Read the model definition and answer for the solid it produces. Units are mm, in the model's axes. A direction names the side the tool comes from. Coordinates: 2 decimals unless noted, no trailing zeros. Write each loop counter-clockwise with the first axis right and the second up, starting at its lowest first coordinate (ties: lowest second). Pieces come first, ordered by that corner, then holes. Notation, with made-up numbers: M 22.25,25.25 L 75.25,25.25 A9 ccw 75.25,34.25 Z; hole C 1.25,80 d2. An arc over 180 degrees is marked long. Write item = value, one per line.
from build123d import *

# Parameters (mm, degrees)
SKETCH_1_R                = 21
SKETCH_1_R_2              = 12.5
EXTRUDE_1_DEPTH           = 71
SKETCH_2_R                = 32.5
SKETCH_2_R_2              = 12.5
EXTRUDE_2_DEPTH           = 13
HOLE_WIZARD_1_D           = 5.5
HOLE_WIZARD_1_CBORE_D     = 10
HOLE_WIZARD_1_CBORE_DEPTH = 5.7


with BuildPart() as part:
    # 草图1 → 凸台-拉伸1 (new body)
    with BuildSketch(Plane.XY):
        Circle(SKETCH_1_R)
        Circle(SKETCH_1_R_2, mode=Mode.SUBTRACT)
    extrude(amount=EXTRUDE_1_DEPTH)

    # 草图2 → 凸台-拉伸2 (add)
    with BuildSketch(Plane(origin=(0, 0, 0), x_dir=(-1, 0, 0), z_dir=(0, 0, -1))):
        Circle(SKETCH_2_R)
        with Locations(Location((0, 0, 0), (0, 0, 180))):
            Circle(SKETCH_2_R_2, mode=Mode.SUBTRACT)
    extrude(amount=-EXTRUDE_2_DEPTH)

    # 打孔尺寸(%根据)内六角圆柱头螺钉的类型1 (through all)
    with Locations(Plane(origin=(0, 26, 0), x_dir=(-1, 0, 0), z_dir=(0, 0, -1))):
        with Locations((0, 0), (26, -26), (0, -52), (-26, -26)):
            CounterBoreHole(HOLE_WIZARD_1_D / 2, HOLE_WIZARD_1_CBORE_D / 2, HOLE_WIZARD_1_CBORE_DEPTH)


solid = part.part
Item 1: Find section B-B (x = -26). Determine the outline of the cut face in (y, z), and give its area (3 significant figures).
Worked answers:
outline = M -19.5,0 L -5,0 L -5,5.7 L -2.75,5.7 L -2.75,13 L -19.5,13 Z; M 2.75,5.7 L 5,5.7 L 5,0 L 19.5,0 L 19.5,13 L 2.75,13 Z
area = 410 mm²
Item 2: Consider line 1 along Y through (x, z) = (0, 3); line 2 along Y through (x, z) = (0, 9.5); line 3 along Z through (x, y) = (15, 25.5). Determine where each line is inside the solid, lowest interval first. Write a range as from..to.
Worked answers:
line_1 = -32.5..-31, -21..-12.5, 12.5..21, 31..32.5
line_2 = -32.5..-28.75, -23.25..-12.5, 12.5..23.25, 28.75..32.5
line_3 = 0..13
Item 3: Which of the six approach directions +Z, -Z, +X, -X, +Y, -Y give full straight-line access (tool end or side, diameter ignored) to faces 1 (the face through (15, 15, 13)), 2 (the face through (1.08, 21.12, 2.81)), 3 (the face through (23.253, 0.121, 9.401))?
Worked answers:
face_1 = +Z
face_2 = -Z
face_3 = +Z, -Z
Item 4: Find section A-A (x = 0). Determine the outline of the cut face in (y, z), and give its area (3 significant figures).
Worked answers:
outline = M -32.5,0 L -31,0 L -31,5.7 L -28.75,5.7 L -28.75,13 L -32.5,13 Z; M -23.25,5.7 L -21,5.7 L -21,0 L -12.5,0 L -12.5,71 L -21,71 L -21,13 L -23.25,13 Z; M 12.5,0 L 21,0 L 21,5.7 L 23.25,5.7 L 23.25,13 L 21,13 L 21,71 L 12.5,71 Z; M 28.75,5.7 L 31,5.7 L 31,0 L 32.5,0 L 32.5,13 L 28.75,13 Z
area = 1,310 mm²
Item 5: Flat-ended cylindrical pins translate along their axes: pin 1 (2 mm diameter, centred on y = 4.5, z = 52, fed in from +X); pin 2 (7 mm diameter, centred on x = -26, y = 0, fed in from -Z); pin 3 (1.5 mm diameter, centred on x = 4.5, z = 17, fed in from +Y). Find the tip coordinate at first contact, or state that the pin passes through.
Worked answers:
pin_1 = 20.71
pin_2 = 5.7
pin_3 = 20.66
Item 6: For a pull along Y with two mould halves and no side action, classify faces 4 (the face through (-14, 0, 0)), 5 (the face through (-21, 0, 3)), 6 (the face through (20.03, 6.31, 41.59)) as released by +Y, released by -Y, zero draft, split by the parting line, or undercut.
Worked answers:
face_4 = zero draft
face_5 = undercut
face_6 = split by the parting line
